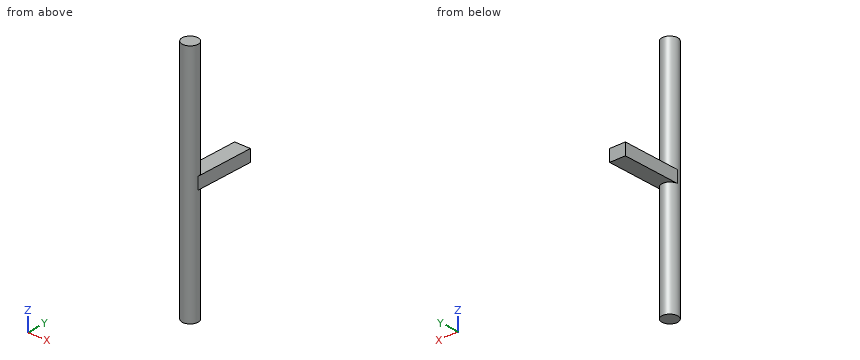
```python
from build123d import *

# Parameters (mm, degrees)
SKETCH1_R           = 4
BOSS_EXTRUDE1_DEPTH = 120
SKETCH2_W           = 8
SKETCH2_H           = 6
BOSS_EXTRUDE2_DEPTH = 30


with BuildPart() as part:
    # Sketch1 → Boss-Extrude1 (new body)
    with BuildSketch(Plane.XY):
        with Locations(Location((0, 0, 0), (0, 0, 180))):
            Circle(SKETCH1_R)
    extrude(amount=BOSS_EXTRUDE1_DEPTH)

    # Sketch2 → Boss-Extrude2 (add)
    with BuildSketch(Plane(origin=(0, 0, 0), x_dir=(1, 0, 0), z_dir=(0, 1, 0))):
        with Locations((0, -60)):
            Rectangle(SKETCH2_W, SKETCH2_H)
    extrude(amount=BOSS_EXTRUDE2_DEPTH)


solid = part.part
```
The listing builds one solid part. Answer for the finished solid, in the listing's coordinates (mm). Give positions to 0.01 mm unless a question says otherwise; leave off trailing zeros. Order: outer loops, then holes, each group sorted by start corner. A loop starts at its lowest first (then second) coordinate and runs counter-clockwise, first axis right, second up. Notation, with made-up numbers: M 25.25,-18 L 59.25,-18 A18 cw 59.25,11 Z; hole C 32.25,40 d9. An arc over 180 degrees is marked long. Put each result on its own line as item: value. Start each with the question number.
Item 1: The part is cut by section B-B, the plane y = 7.5. Determine the outline of the cut face in (x, z).
Item 2: The part is cut by section A-A, the plane x = 0. Determine the outline of the cut face in (y, z).
Item 3: Flat-ended cylindrical pins translate along their axes: P1, Ø1.5, axis at x = -2.5, y = 9.5, coming from the -Z side; P2, Ø6, axis at y = 18.5, z = 67.5, coming from the -X side; P3, Ø3, axis at y = 2.5, z = 26.5, coming from the -X side. Find the tip coordinate at first contact, or state that the pin passes through.
Item 4: The part is cut by section D-D, the plane y = 3. Determine the outline of the cut face in (x, z).
Item 5: Find the intervals of material crossed by line 1 along Z through (x, y) = (3, 27); line 2 along Y through (x, z) = (0, 49.5); line 3 along Y through (x, z) = (-3, 69), in increasing order.
Item 6: The part is cut by section C-C, the plane z = 65. Determine the outline of the cut face in (x, y), and give its area (3 significant figures).
Answer key:
1. outline: M -4,57 L 4,57 L 4,63 L -4,63 Z
2. outline: M -4,0 L 4,0 L 4,57 L 30,57 L 30,63 L 4,63 L 4,120 L -4,120 Z
3. P1: stops at z = 57
3. P2: passes through
3. P3: stops at x = -3.87
4. outline: M -4,57 L -2.65,57 L -2.65,0 L 2.65,0 L 2.65,57 L 4,57 L 4,63 L 2.65,63 L 2.65,120 L -2.65,120 L -2.65,63 L -4,63 Z
5. line 1: z = 57 to 63
5. line 2: y = -4 to 4
5. line 3: y = -2.65 to 2.65
6. outline: C 0,0 d8
6. area: 50.3 mm²
